from build123d import *

# Parameters (mm, degrees)
EXTRUDE_1_DEPTH = 529


with BuildPart() as part:
    # 草图1 → 凸台-拉伸1 (new, symmetric)
    with BuildSketch(Plane.XY):
        with BuildLine():
            Line((-4.556913863, 4.138102128), (-2.645672962, 1.79891143))
            Line((-2.645672962, 1.79891143), (-5, 1.79891143))
            Line((-5, 1.79891143), (-5, 1.29891143))
            Line((-5, 1.29891143), (1.591473901, 1.29891143))
            Line((1.591473901, 1.29891143), (5, 1.29891143))
            Line((5, 1.29891143), (5, 1.79891143))
            Line((5, 1.79891143), (2.645672962, 1.79891143))
            Line((2.645672962, 1.79891143), (4.556913863, 4.138102128))
            ThreePointArc((4.556913863, 4.138102128), (4.780792009, 4.829714088), (4.47713902, 5.490201325))
            ThreePointArc((4.47713902, 5.490201325), (0, 7.29891143), (-4.47713902, 5.490201325))
            ThreePointArc((-4.47713902, 5.490201325), (-4.780792009, 4.829714088), (-4.556913863, 4.138102128))
        make_face()
        with BuildLine():
            Line((-2, 1.79891143), (2, 1.79891143))
            Line((2, 1.79891143), (4.169720942, 4.454458955))
            ThreePointArc((4.169720942, 4.454458955), (4.281660015, 4.800264935), (4.12983352, 5.130508554))
            ThreePointArc((4.12983352, 5.130508554), (0, 6.79891143), (-4.12983352, 5.130508554))
            ThreePointArc((-4.12983352, 5.130508554), (-4.281660015, 4.800264935), (-4.169720942, 4.454458955))
            Line((-4.169720942, 4.454458955), (-2, 1.79891143))
        make_face(mode=Mode.SUBTRACT)
    extrude(amount=EXTRUDE_1_DEPTH, both=True)


solid = part.part
For this review, take the finished solid that the model builds, in its own axes (mm). Give positions to 0.01 mm unless a question says otherwise; leave off trailing zeros. Order: outer loops, then holes, each group sorted by start corner. A loop starts at its lowest first (then second) coordinate and runs counter-clockwise, first axis right, second up. Notation, with made-up numbers: (82.5, -24.5) -> (136.5, -24.5) arc R5 cw to (136.5, -17.5) -> close; hole circle Ø6 at (57.5, 71.25). An arc over 180 degrees is marked (long way). Write item = value, one per line.
1) To check wall thickness, follow L1, parallel to X at y = 4.7, z = -376; L2, parallel to Y at x = 3.75, z = 232; L3, parallel to Y at x = -0.25, z = -339. State the ranges of each line that lie inside material, in increasing order. Write a range as from..to.
Findings:
L1 = -4.78..-4.28, 4.28..4.78
L2 = 1.3..1.8, 3.15..3.94, 5.47..6.1
L3 = 1.3..1.8, 6.79..7.29
2) We need section B-B, the plane z = 41. Give the boundary of the cut face in (x, y), and give its area (3 significant figures).
Findings:
outline = (-5, 1.3) -> (5, 1.3) -> (5, 1.8) -> (2.65, 1.8) -> (4.56, 4.14) arc R1 ccw to (4.48, 5.49) arc R6.45 ccw to (-4.48, 5.49) arc R1 ccw to (-4.56, 4.14) -> (-2.65, 1.8) -> (-5, 1.8) -> close; hole (-4.17, 4.45) -> (-2, 1.8) -> (2, 1.8) -> (4.17, 4.45) arc R0.5 ccw to (4.13, 5.13) arc R5.95 ccw to (-4.13, 5.13) arc R0.5 ccw to start
area = 14.1 mm^2
3) Insertion check: pin 1 (1.2 mm diameter, centred on x = 4, z = 89, fed in from +Y); pin 2 (2.5 mm diameter, centred on x = -4, z = -58, fed in from +Y). Each pin has a flat end and moves straight along its axis. Give the tip position at first contact, or say it passes through.
Findings:
pin_1 = 6.33
pin_2 = 6.68
4) We need section A-A, the plane x = -0.25. Give the boundary of the cut face in (y, z).
Findings:
outline = (1.3, -529) -> (1.8, -529) -> (1.8, 529) -> (1.3, 529) -> close; (6.79, -529) -> (7.29, -529) -> (7.29, 529) -> (6.79, 529) -> close
